For this review, use the dimensioned drawing (mm, ordinates from the lowest corner) and the shaded views. A direction names the side the tool comes from. Coordinates: 2 decimals unless noted, no trailing zeros. Loops run counter-clockwise (first coordinate to the right, second up) from the corner with the lowest first, then second, coordinate; pieces in that order, holes last. Notation, with made-up numbers: (31.5, 68.5) -> (60.5, 68.5) arc R21 ccw to (60.5, 77.5) -> close; hole circle Ø4 at (45, -13.75). An arc over 180 degrees is marked (long way). Use one line per item in the form item = value. Start each with the question number.
1. Consider section B-B (y = 10). State the section outline as (x, z) points, then the cut area to 3 significant figures.
2. Wall thickness on line 1 (X direction, y = 10, z = 11); line 2 (X direction, y = 2.25, z = 12); line 3 (X direction, y = 11.75, z = 13.25): over which ranges is each line inside the solid? List them lowest first. Write a range as from..to.
3. Consider section D-D (x = 7.25). State the section outline as (y, z) points, then the cut area to 3 significant figures.
4. Consider section C-C (x = 22). State the section outline as (y, z) points, then the cut area to 3 significant figures.
5. For pin 1 (3 mm diameter, centred on x = 3, y = 7, fed in from -Z); pin 2 (1.5 mm diameter, centred on x = 10.5, z = 14.5, fed in from -Y); pin 3 (10 mm diameter, centred on x = 13.5, y = 8, fed in from -Z), all flat-tipped, find the tip position at first contact; note any pin that passes through.
6. Machinability: for the marked faces 5 and 6, which of the approach directions +Z, -Z, +X, -X, +Y, -Y give a long, thin tool a straight path to every point of the face, cutting with its end or side? Answer none if there is none.
7. Consider section A-A (z = 10). State the section outline as (x, y) points, then the cut area to 3 significant figures.
8. The part is to be moulded in two halves that separate along X. For the marked faces 1, 2, 3 and 4, say which applies: released by +X, released by -X, zero draft, split by the parting line, or undercut.
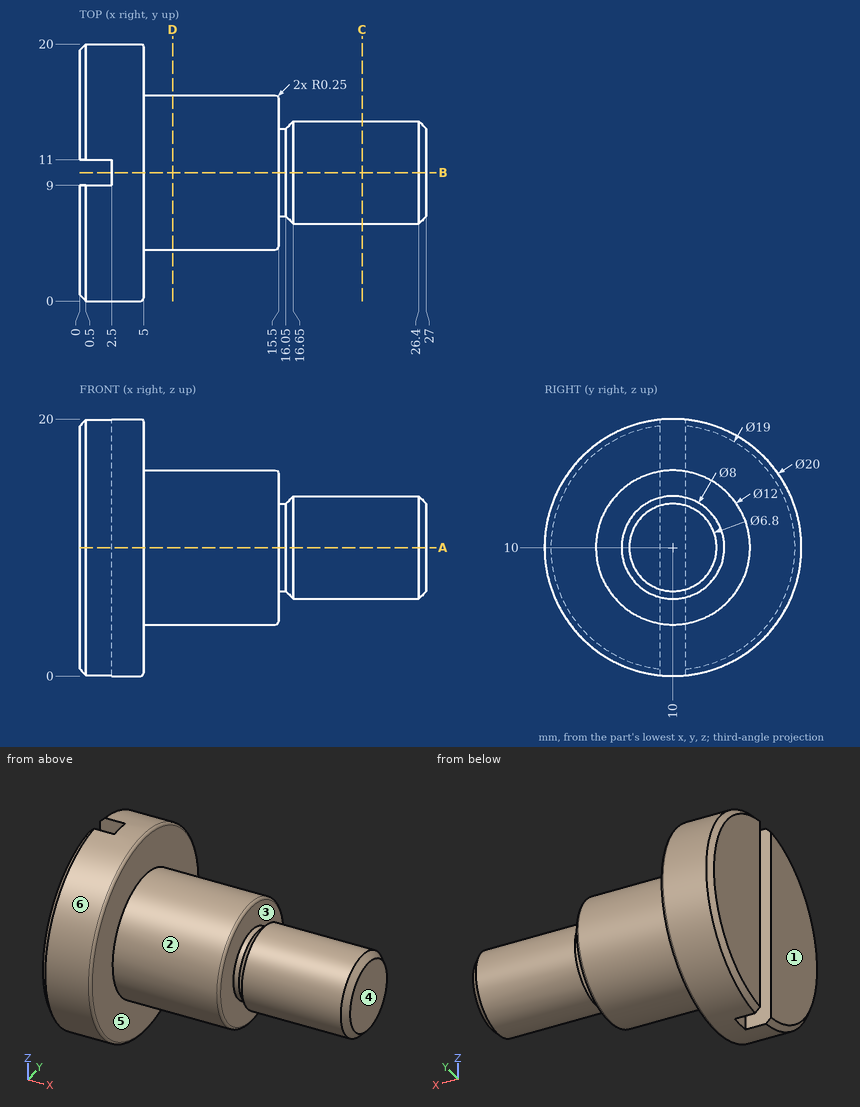
Geometry check:
q1.outline = (2.5, 0) -> (4.75, 0) arc R0.25 ccw to (5, 0.25) -> (5, 4) -> (15.25, 4) arc R0.25 ccw to (15.5, 4.25) -> (15.5, 6.6) -> (16.05, 6.6) -> (16.65, 6) -> (26.4, 6) -> (27, 6.6) -> (27, 13.4) -> (26.4, 14) -> (16.65, 14) -> (16.05, 13.4) -> (15.5, 13.4) -> (15.5, 15.75) arc R0.25 ccw to (15.25, 16) -> (5, 16) -> (5, 19.75) arc R0.25 ccw to (4.75, 20) -> (2.5, 20) -> close
q1.area = 267 mm²
q2.line_1 = 2.5..27
q2.line_2 = 0..5
q2.line_3 = 0..15.5, 16.34..26.71
q3.outline = circle Ø12 at (10, 10)
q3.area = 113 mm²
q4.outline = circle Ø8 at (10, 10)
q4.area = 50.3 mm²
q5.pin_1 = 0.11
q5.pin_2 = 5.32
q5.pin_3 = 4
q6.face_5 = +X
q6.face_6 = +X, -X
q7.outline = (0, 0.5) -> (0.5, 0) -> (4.75, 0) arc R0.25 ccw to (5, 0.25) -> (5, 4) -> (15.25, 4) arc R0.25 ccw to (15.5, 4.25) -> (15.5, 6.6) -> (16.05, 6.6) -> (16.65, 6) -> (26.4, 6) -> (27, 6.6) -> (27, 13.4) -> (26.4, 14) -> (16.65, 14) -> (16.05, 13.4) -> (15.5, 13.4) -> (15.5, 15.75) arc R0.25 ccw to (15.25, 16) -> (5, 16) -> (5, 19.75) arc R0.25 ccw to (4.75, 20) -> (0.5, 20) -> (0, 19.5) -> (0, 11) -> (2.5, 11) -> (2.5, 9) -> (0, 9) -> close
q7.area = 311 mm²
q8.face_1 = released by -X
q8.face_2 = zero draft
q8.face_3 = undercut
q8.face_4 = released by +X
